```python
from build123d import *

# Parameters (mm, degrees)
SKETCH3_W           = 130
SKETCH3_H           = 80
BOSS_EXTRUDE1_DEPTH = 10
SKETCH4_W           = 8
SKETCH4_H           = 80
BOSS_EXTRUDE2_DEPTH = 5


with BuildPart() as part:
    # Sketch3 → Boss-Extrude1 (new body)
    with BuildSketch(Plane.XY):
        with Locations((720, 119)):
            Rectangle(SKETCH3_W, SKETCH3_H)
    extrude(amount=BOSS_EXTRUDE1_DEPTH)

    # Sketch4 → Boss-Extrude2 (add)
    with BuildSketch(Plane(origin=(0, 0, 0), x_dir=(-1, 0, 0), z_dir=(0, 0, -1))):
        with Locations((-735, 119)):
            Rectangle(SKETCH4_W, SKETCH4_H)
        with Locations((-705, 119)):
            Rectangle(SKETCH4_W, SKETCH4_H)
    extrude(amount=BOSS_EXTRUDE2_DEPTH)


solid = part.part
```
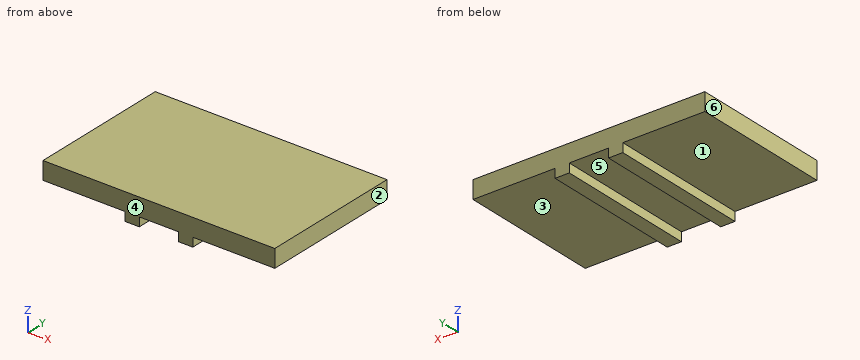
Geometry: final body of the model. Coordinates: model frame, mm. Face numbers are marked on the shaded views. A direction names the side the tool comes from. Give positions to 0.01 mm unless a question says otherwise; leave off trailing zeros. Loops run counter-clockwise (first coordinate to the right, second up) from the corner with the lowest first, then second, coordinate; pieces in that order, holes last. Notation, with made-up numbers: (52.25, 53.25) -> (56.25, 53.25) arc R26 ccw to (56.25, 69.25) -> close; hole circle Ø5 at (-37, 58). An arc over 180 degrees is marked (long way). Use CSV: the item, a comma, the result in double quotes.
(1) Pull-direction query (X, two-part tool) for the marked faces 4, 5 and 6; classes: released by +X, released by -X, zero draft, split by the parting line, or undercut.
From the geometry:
face 4,"zero draft"
face 5,"undercut"
face 6,"released by -X"
(2) Cut plane A-A (z = -2.5). Output: boundary loops of the cut face in (x, y), plus the area to 3 significant figures.
From the geometry:
outline,"(701, 79) -> (709, 79) -> (709, 159) -> (701, 159) -> close; (731, 79) -> (739, 79) -> (739, 159) -> (731, 159) -> close"
area,"1,280 mm^2"
(3) Ray query, line 1 along X through (y, z) = (91, -0.5); line 2 along Z through (x, y) = (728, 114). Return the intervals inside material, ascending. Write a range as [from, to].
From the geometry:
line 1,"[701, 709], [731, 739]"
line 2,"[0, 10]"
(4) Access query for the marked faces 1, 2 and 3. Directions: +Z, -Z, +X, -X, +Y, -Y. A direction counts if a zero-diameter tool reaches every point of the face in a straight line with its end or side. Return the directions, or none.
From the geometry:
face 1,"-Z, -X, +Y, -Y"
face 2,"+Z, -Z, +X, +Y, -Y"
face 3,"-Z, +X, +Y, -Y"
(5) Cut plane C-C (x = 749). Output: boundary loops of the cut face in (y, z), plus the area to 3 significant figures.
From the geometry:
outline,"(79, 0) -> (159, 0) -> (159, 10) -> (79, 10) -> close"
area,"800 mm^2"
(6) First-contact query: P1, Ø5, axis at y = 119, z = -2, coming from the -X side; P2, Ø1.5, axis at y = 104.5, z = -3, coming from the -X side; P3, Ø11, axis at x = 725, y = 124.5, coming from the -Z side; P4, Ø2.5, axis at y = 125.5, z = -3, coming from the +X side. Flat tips, straight axial feed; report the tip coordinate or a pass-through.
From the geometry:
P1,"x = 655"
P2,"x = 701"
P3,"z = 0"
P4,"x = 739"
(7) Cut plane B-B (y = 101.5). Output: boundary loops of the cut face in (x, z).
From the geometry:
outline,"(655, 0) -> (701, 0) -> (701, -5) -> (709, -5) -> (709, 0) -> (731, 0) -> (731, -5) -> (739, -5) -> (739, 0) -> (785, 0) -> (785, 10) -> (655, 10) -> close"
